Design review of the part shown in the three views and the two pictorial views. Dimensions are in mm from the part's minimum x, y and z. Coordinates: 2 decimals unless noted, no trailing zeros. Loops run counter-clockwise (first coordinate to the right, second up) from the corner with the lowest first, then second, coordinate; pieces in that order, holes last. Notation, with made-up numbers: (47, 15.5) - (95, 15.5) arc R22 cw to (95, 37.5) - close; hole circle Ø2 at (37, 36.25). An arc over 180 degrees is marked (long way). One line per item, written item: value. Start each with the question number.
1. Take a section at A-A, the plane y = 35. State the section outline as (x, z) points, and give its area (3 significant figures).
2. To check wall thickness, follow line 1 (Y direction, x = 180, z = 8.25); line 2 (Y direction, x = 16, z = 11). State the ranges of each line that lie inside material, in increasing order. Write a range as from..to.
3. Take a section at C-C, the plane x = 178. State the section outline as (y, z) points.
4. Take a section at B-B, the plane x = 20. State the section outline as (y, z) points.
5. Insertion check: pin 1 (8 mm diameter, centred on x = 20, y = 35, fed in from +Z). The pin has a flat end and moves straight along its axis. Give the tip position at first contact, or say it passes through.
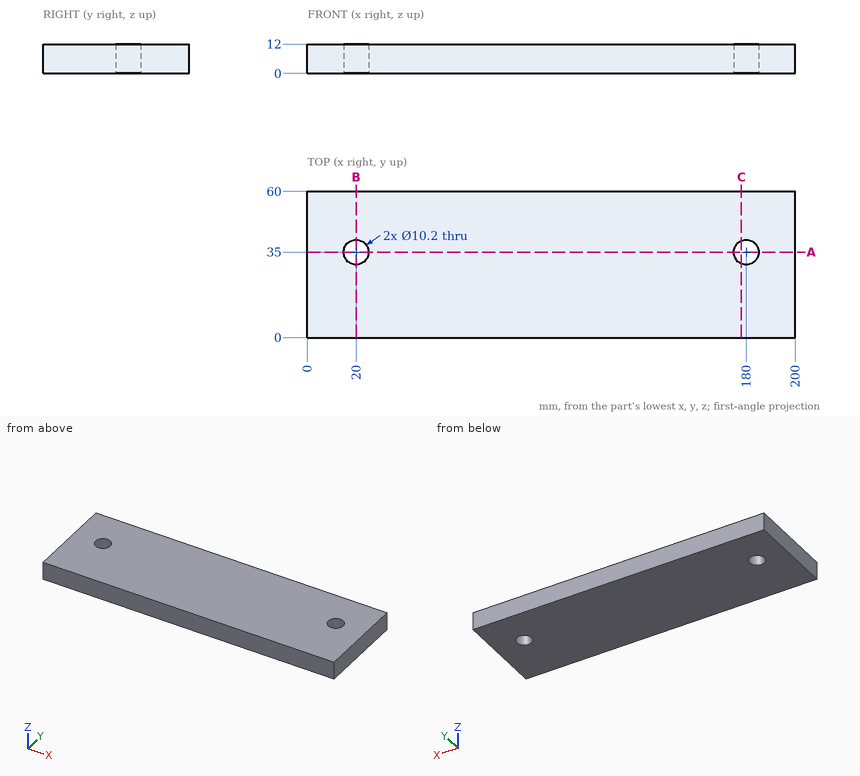
Solutions:
1. outline: (0, 0) - (14.9, 0) - (14.9, 12) - (0, 12) - close; (25.1, 0) - (174.9, 0) - (174.9, 12) - (25.1, 12) - close; (185.1, 0) - (200, 0) - (200, 12) - (185.1, 12) - close
1. area: 2,160 mm2
2. line 1: 0..29.9, 40.1..60
2. line 2: 0..31.84, 38.16..60
3. outline: (0, 0) - (30.31, 0) - (30.31, 12) - (0, 12) - close; (39.69, 0) - (60, 0) - (60, 12) - (39.69, 12) - close
4. outline: (0, 0) - (29.9, 0) - (29.9, 12) - (0, 12) - close; (40.1, 0) - (60, 0) - (60, 12) - (40.1, 12) - close
5. pin 1: through
